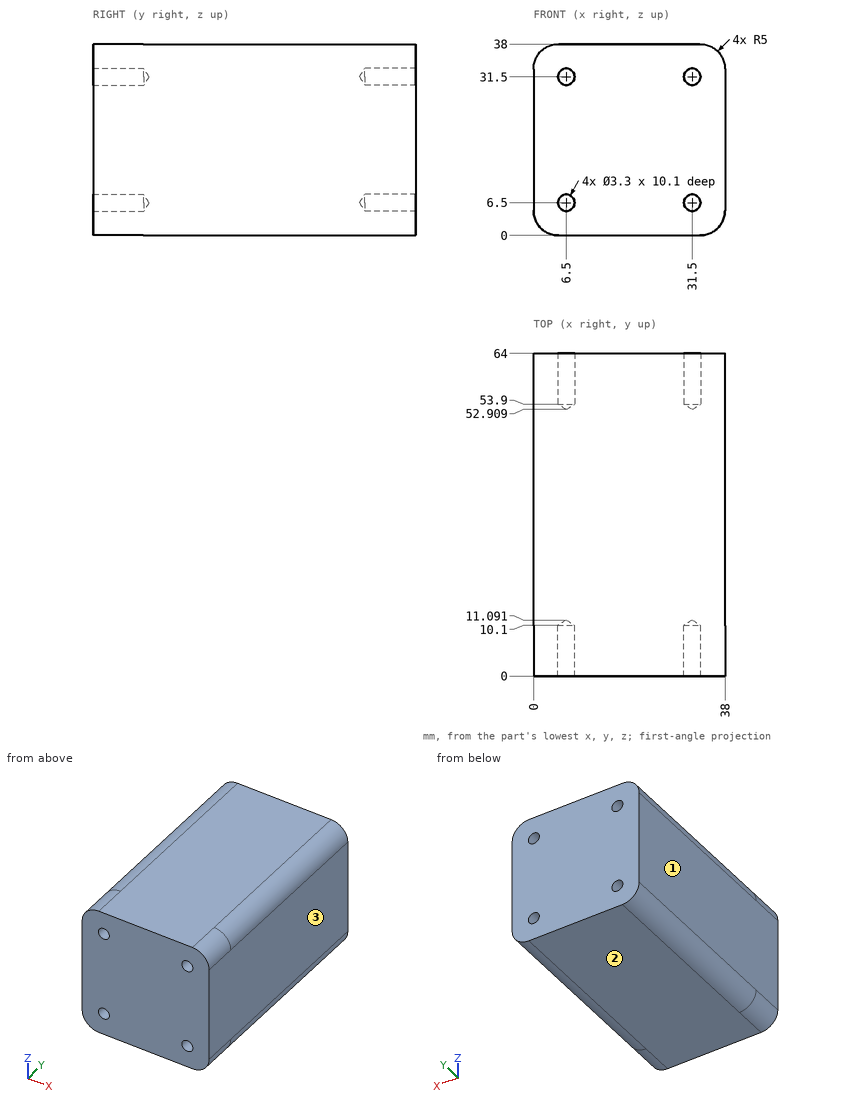
Print and shaded views of the part. All mm, measured from the part's lowest x, y and z. Round coordinates to 2 decimals unless told otherwise and drop trailing zeros. One line per item, written item: value.
(1) Drop flat-ended pins along their axis: P1, Ø5.5, axis at x = 6.5, z = 6.5, coming from the -Y side; P2, Ø3, axis at x = 6.5, z = 31.5, coming from the +Y side; P3, Ø2.5, axis at x = 31.5, z = 31.5, coming from the +Y side; P4, Ø2, axis at x = 31.5, z = 6.5, coming from the +Y side. Give the stop position or say it passes through.
Values follow:
P1: stops at y = 0
P2: stops at y = 53.81
P3: stops at y = 53.66
P4: stops at y = 53.51
(2) Wall check: probe 1 along Z at (x, y) = (6.5, 58.75); probe 2 along X at (y, z) = (56, 31). Give the ranges that are in metal, low to high.
Values follow:
probe 1: z = 0 to 4.85, 8.15 to 29.85, 33.15 to 38
probe 2: x = 0 to 4.93, 8.07 to 29.93, 33.07 to 38
(3) Two-plate mould, pull along X, no slides. Class the marked faces 1, 2 and 3: pulls with the +X half, pulls with the -X half, needs draft (parallel to the pull), parting line crosses it, or undercut.
Values follow:
face 1: pulls with the -X half
face 2: needs draft
face 3: pulls with the +X half
